Design review of the part built by this model. Coordinates are the model's own, in mm. A direction names the side the tool comes from. Coordinates: 2 decimals unless noted, no trailing zeros.
Q1. The part is to be moulded in two halves that separate along Z. For faces 1 (the face through (0, 14, -17)), 2 (the face through (375, 14, -34)), 3 (the face through (584.73, 23.08, -22.16)), say which applies: +Z half, -Z half, draft (parallel to the pull), parting line (faces both ways), or undercut.
Q2. Clearance check with flat-ended pins moving along their axes: pin 1 Ø15.5 at (x, z) = (580, -19) entering from +Y; pin 2 Ø11.5 at (x, z) = (580, -17) entering from +Y. State where each tip first meets the part, or that it passes through.
Q3. Add section A-A, the plane y = 7.5. Give the number of separate pieces and of enclosed holes in the cut face, plus the area to 3 significant figures.
Q4. Machinability: for faces 4 (the face through (173.166, 23.084, -18.517)), 5 (the face through (760, 14, -17)), which of the approach directions +Z, -Z, +X, -X, +Y, -Y give a long, thin tool a straight path to every point of the face, cutting with its end or side? Answer none if there is none.
Q5. To check wall thickness, follow probe 1 along Z at (x, y) = (340, 10.5); probe 2 along Y at (x, z) = (501, -22); probe 3 along Z at (x, y) = (97, 9.25). State the ranges of each line that lie inside material, in increasing order.
from build123d import *

# Parameters (mm, degrees)
SKETCH_1_W             = 760
SKETCH_1_H             = 34
EXTRUDE_1_DEPTH        = 29
SKETCH_2_R             = 7
CUT_EXTRUDE_1_DEPTH    = 12
SKETCH_3_R             = 4.5
CUT_EXTRUDE_2_DEPTH    = 761.950064065
PATTERN_LINEAR_1_COUNT = 10
PATTERN_LINEAR_1_PITCH = 80


with BuildPart() as part:
    # 草图1 → 拉伸1 (new body)
    with BuildSketch(Plane(origin=(0, 0, 0), x_dir=(1, 0, 0), z_dir=(0, 1, 0))):
        with Locations((380, 17)):
            Rectangle(SKETCH_1_W, SKETCH_1_H)
    extrude(amount=EXTRUDE_1_DEPTH)

    # 草图2 → 切除-拉伸1 (cut)
    with BuildSketch(Plane(origin=(0, 29, 0), x_dir=(-1, 0, 0), z_dir=(0, 1, 0))):
        with Locations(Location((-20, -17, 0), (0, 0, 90))):
            Circle(SKETCH_2_R)
    cut_extrude_1 = extrude(amount=-CUT_EXTRUDE_1_DEPTH, mode=Mode.SUBTRACT)

    # 草图3 → 切除-拉伸2 (cut, through all)
    with BuildSketch(Plane(origin=(0, 17, 0), x_dir=(-1, 0, 0), z_dir=(0, 1, 0))):
        with Locations(Location((-20, -17, 0), (0, 0, 90))):
            Circle(SKETCH_3_R)
    cut_extrude_2 = extrude(amount=-CUT_EXTRUDE_2_DEPTH, mode=Mode.SUBTRACT)

    # 阵列(线性)1: 切除-拉伸1, 切除-拉伸2 ×10
    with Locations(*[(i * PATTERN_LINEAR_1_PITCH, 0, 0) for i in range(1, PATTERN_LINEAR_1_COUNT)]):
        add(cut_extrude_1, mode=Mode.SUBTRACT)
        add(cut_extrude_2, mode=Mode.SUBTRACT)


solid = part.part
Here are the results:
1. face 1: draft
1. face 2: -Z half
1. face 3: undercut
2. pin 1: stops at y = 29
2. pin 2: stops at y = 17
3. separate pieces: 1
3. enclosed holes: 10
3. area: 25,200 mm2
4. face 4: +Y
4. face 5: +Z, -Z, +X, +Y, -Y
5. probe 1: z = -34 to -21.5, -12.5 to 0
5. probe 2: y = 0 to 17
5. probe 3: z = -34 to -20.35, -13.65 to 0
